from build123d import *

# Parameters (mm, degrees)
BOSS_EXTRUDE1_DEPTH                                  = 8
HOLE_SIZE_PER_SOCKET_HEAD_CAP_SCREW_TYPE_D           = 4.5
HOLE_SIZE_PER_SOCKET_HEAD_CAP_SCREW_TYPE_CBORE_D     = 8
HOLE_SIZE_PER_SOCKET_HEAD_CAP_SCREW_TYPE_CBORE_DEPTH = 4.6


with BuildPart() as part:
    # Sketch1 → Boss-Extrude1 (new body)
    with BuildSketch(Plane.XY):
        with BuildLine():
            Line((-30.0520382, -12.374368671), (-12.374368671, -30.0520382))
            ThreePointArc((-12.374368671, -30.0520382), (0, -32.5), (12.374368671, -30.0520382))
            Line((12.374368671, -30.0520382), (30.0520382, -12.374368671))
            ThreePointArc((30.0520382, -12.374368671), (32.5, 0), (30.0520382, 12.374368671))
            Line((30.0520382, 12.374368671), (12.374368671, 30.0520382))
            ThreePointArc((12.374368671, 30.0520382), (0, 32.5), (-12.374368671, 30.0520382))
            Line((-12.374368671, 30.0520382), (-30.0520382, 12.374368671))
            ThreePointArc((-30.0520382, 12.374368671), (-32.5, 0), (-30.0520382, -12.374368671))
        make_face()
    extrude(amount=BOSS_EXTRUDE1_DEPTH)

    # Hole size per socket head cap screw type 1 (through all)
    with Locations(Plane.XY.offset(8)):
        with Locations((0, 27.5), (-27.5, 0), (0, -27.5), (27.5, 0)):
            CounterBoreHole(HOLE_SIZE_PER_SOCKET_HEAD_CAP_SCREW_TYPE_D / 2, HOLE_SIZE_PER_SOCKET_HEAD_CAP_SCREW_TYPE_CBORE_D / 2, HOLE_SIZE_PER_SOCKET_HEAD_CAP_SCREW_TYPE_CBORE_DEPTH)


solid = part.part
Source: CAD feature listing. Evaluate the final solid. Frame: model axes, mm. A direction names the side the tool comes from. Coordinates: 2 decimals unless noted, no trailing zeros. Order: outer loops, then holes, each group sorted by start corner. A loop starts at its lowest first (then second) coordinate and runs counter-clockwise, first axis right, second up. Notation, with made-up numbers: M 63,57 L 96,57 A15 ccw 96,63 Z; hole C -28,58 d10. An arc over 180 degrees is marked long. Write each question's results on one line, items separated by ' | '. Start each with the question number.
1. Draft query along Y for faces 1 (the face through (2, -29, 3.4)), 2 (the face through (0.2, 32.5, 3.9)), 3 (the face through (-21.337, -21.089, 3.944)). Return one class per face: +Y half, -Y half, draft (parallel to the pull), parting line (faces both ways), or undercut.
2. Pin query (flat end, axial travel): pin 1 (4 mm diameter, centred on x = 1, y = -28.5, fed in from +Z); pin 2 (1 mm diameter, centred on x = -20, z = 1, fed in from -Y); pin 3 (1 mm diameter, centred on y = 11.5, z = 4.5, fed in from +X); pin 4 (4 mm diameter, centred on x = 27.5, y = 0, fed in from +Z). Return the tip coordinate at first contact, or that it passes through.
3. Reachability of faces 4 (the face through (0, 0, 0)), 5 (the face through (-26, -2, 3.4)) from +Z, -Z, +X, -X, +Y, -Y: full face, straight path, thin tool, end or side. Return the list, or none.
4. Section A-A, the plane x = 0. Return the cut outline in (y, z), then the cut area to 3 significant figures.
5. Section C-C, the plane y = -26. Return the cut outline in (x, z), then the cut area to 3 significant figures.
6. Material intervals for L1, parallel to Y at x = 0, z = 6.35; L2, parallel to Y at x = -1, z = 2.5; L3, parallel to Y at x = 27.5, z = 1.3, sorted ascending.
Solution:
1) face 1: undercut | face 2: +Y half | face 3: -Y half
2) pin 1: z = 3.4 | pin 2: y = -22.93 | pin 3: x = 30.58 | pin 4: through
3) face 4: -Z, +X, -X, +Y, -Y | face 5: +Z
4) outline: M -32.5,0 L -29.75,0 L -29.75,3.4 L -31.5,3.4 L -31.5,8 L -32.5,8 Z; M -25.25,0 L 25.25,0 L 25.25,3.4 L 23.5,3.4 L 23.5,8 L -23.5,8 L -23.5,3.4 L -25.25,3.4 Z; M 29.75,0 L 32.5,0 L 32.5,8 L 31.5,8 L 31.5,3.4 L 29.75,3.4 Z | area: 416 mm²
5) outline: M -16.43,0 L -1.68,0 L -1.68,3.4 L -3.71,3.4 L -3.71,8 L -16.43,8 Z; M 1.68,0 L 16.43,0 L 16.43,8 L 3.71,8 L 3.71,3.4 L 1.68,3.4 Z | area: 217 mm²
6) L1: -32.5 to -31.5, -23.5 to 23.5, 31.5 to 32.5 | L2: -32.48 to -29.52, -25.48 to 25.48, 29.52 to 32.48 | L3: -14.93 to -2.25, 2.25 to 14.93
